Input: part model. Units: mm. Frame: model coordinates. A direction names the side the tool comes from. Give positions to 0.01 mm unless a question says otherwise; leave off trailing zeros. Loops run counter-clockwise (first coordinate to the right, second up) from the corner with the lowest first, then second, coordinate; pieces in that order, holes last. Notation, with made-up numbers: M -20.75,37.25 L 25.25,37.25 A30 ccw 25.25,70.25 Z; hole C 56.5,45.25 d7. An arc over 180 degrees is marked long. Answer as a JSON object with one key per item and string values. Group by question number.
1) Access query for faces 4 (the flat face through (2, 0, 23)), 5 (the flat face through (-6, 0, 13)), 6 (the cylindrical face through (0.27, -1.22, 18.35)). Directions: +Z, -Z, +X, -X, +Y, -Y. A direction counts if a zero-diameter tool reaches every point of the face in a straight line with its end or side. Return the directions, or none.
2) Ray query, L1, parallel to Y at x = 0, z = 8.5; L2, parallel to Y at x = 0, z = 18.75; L3, parallel to Z at x = 0, y = 9. Return the intervals inside material, ascending.
3) Draft query along Y for faces 1 (the flat face through (-3.042, 5.172, 12.528)), 2 (the conical face through (-26.85, -8.45, 0.15)), 3 (the flat face through (0, -23, 0)). Return one class per face: +Y half, -Y half, draft (parallel to the pull), parting line (faces both ways), or undercut.
4) Section query B-B on z = 6.75. Return loops of the section in (x, y).
5) First-contact query: P1, Ø3, axis at x = -7, z = 9, coming from the -Y side; P2, Ø5, axis at y = 12, z = 5, coming from the +X side; P3, Ø4, axis at x = 0, y = 0, coming from the +Z side. Flat tips, straight axial feed; report the tip coordinate or a pass-through.
6) Section query C-C on z = 15.25. Return loops of the section in (x, y), plus the area to 3 significant figures.
from build123d import *

# Parameters (mm, degrees)
SKETCH1_R                   = 31
BOSS_EXTRUDE1_DEPTH         = 26
SKETCH2_R                   = 22.5
CUT_EXTRUDE1_DEPTH          = 11
CUT_EXTRUDE2_DEPTH          = 3.1
CUT_EXTRUDE3_START          = -4
SKETCH4_R                   = 22.5
SKETCH4_R_2                 = 8
CUT_EXTRUDE3_DEPTH          = 4
CUT_EXTRUDE4_START          = -3
SKETCH5_R                   = 8
CUT_EXTRUDE4_DEPTH          = 3
M3_TAPPED_HOLE1_D           = 2.5
M3_TAPPED_HOLE1_CSINK_D     = 3.05
M3_TAPPED_HOLE1_CSINK_ANGLE = 90
CHAMFER1_SIZE               = 3


with BuildPart() as part:
    # Sketch1 → Boss-Extrude1 (new body)
    with BuildSketch(Plane.XY):
        with Locations(Location((0, 0, 0), (0, 0, 180))):
            Circle(SKETCH1_R)
    extrude(amount=BOSS_EXTRUDE1_DEPTH)

    # Sketch2 → Cut-Extrude1 (cut)
    with BuildSketch(Plane(origin=(0, 0, 0), x_dir=(-1, 0, 0), z_dir=(0, 0, -1))):
        Circle(SKETCH2_R)
    extrude(amount=-CUT_EXTRUDE1_DEPTH, mode=Mode.SUBTRACT)

    # Sketch3 → Cut-Extrude2 (cut)
    with BuildSketch(Plane(origin=(0, 0, 11), x_dir=(-1, 0, 0), z_dir=(0, 0, -1))):
        Polygon((0, 6.92820323), (-6, 3.464101615), (-6, -3.464101615), (0, -6.92820323), (6, -3.464101615), (6, 3.464101615), align=None)
    extrude(amount=-CUT_EXTRUDE2_DEPTH, mode=Mode.SUBTRACT)

    # Sketch4 → Cut-Extrude3 (cut)
    with BuildSketch(Plane.XY.offset(26).offset(CUT_EXTRUDE3_START)):
        with Locations(Location((0, 0, 0), (0, 0, 180))):
            Circle(SKETCH4_R)
        Circle(SKETCH4_R_2, mode=Mode.SUBTRACT)
    extrude(amount=CUT_EXTRUDE3_DEPTH, mode=Mode.SUBTRACT)

    # Sketch5 → Cut-Extrude4 (cut)
    with BuildSketch(Plane.XY.offset(26).offset(CUT_EXTRUDE4_START)):
        Circle(SKETCH5_R)
    extrude(amount=CUT_EXTRUDE4_DEPTH, mode=Mode.SUBTRACT)

    # M3 Tapped Hole1 (through all)
    with Locations(Plane.XY.offset(23)):
        with Locations((0, 0)):
            CounterSinkHole(M3_TAPPED_HOLE1_D / 2, M3_TAPPED_HOLE1_CSINK_D / 2, counter_sink_angle=M3_TAPPED_HOLE1_CSINK_ANGLE)

    # Chamfer1
    chamfer1_edges = [part.edges().sort_by_distance(p)[0] for p in [
        (31, 0, 0),
        (31, 0, 26),
    ]]
    chamfer(chamfer1_edges, length=CHAMFER1_SIZE)


solid = part.part
Output:
{
 "1": {"face 4": "+Z", "face 5": "-Z", "face 6": "+Z, -Z"},
 "2": {"L1": "y = -31 to -22.5, 22.5 to 31", "L2": "y = -31 to -1.25, 1.25 to 31", "L3": "z = 11 to 22"},
 "3": {"face 1": "undercut", "face 2": "parting line", "face 3": "draft"},
 "4": {"outline": "C 0,0 d62; hole C 0,0 d45"},
 "5": {"P1": "stops at y = -30.51", "P2": "stops at x = 29.51", "P3": "stops at z = 23"},
 "6": {"outline": "C 0,0 d62; hole C 0,0 d2.5", "area": "3,010 mm^2"}
}
